from build123d import *

# Parameters (mm, degrees)
SKETCH1_W           = 220
SKETCH1_H           = 220
BOSS_EXTRUDE1_DEPTH = 70
SKETCH2_R           = 82.5
CUT_EXTRUDE1_DEPTH  = 171.587221092
M30_TAPPED_HOLE1_D  = 26.5
SKETCH7_R           = 22.5
CUT_EXTRUDE3_DEPTH  = 5
FILLET1_R           = 30
CHAMFER1_SIZE       = 3
SKETCH8_W           = 16
SKETCH8_H           = 87
CUT_EXTRUDE4_DEPTH  = 171.587221092


with BuildPart() as part:
    # Sketch1 → Boss-Extrude1 (new body)
    with BuildSketch(Plane.XY):
        Rectangle(SKETCH1_W, SKETCH1_H)
    extrude(amount=BOSS_EXTRUDE1_DEPTH)

    # Sketch2 → Cut-Extrude1 (cut, through all)
    with BuildSketch(Plane.XY.offset(70)):
        Circle(SKETCH2_R)
    extrude(amount=-CUT_EXTRUDE1_DEPTH, mode=Mode.SUBTRACT)

    # M30 Tapped Hole1 (through all)
    with Locations(Plane(origin=(110, 0, 0), x_dir=(0, 0, -1), z_dir=(1, 0, 0))):
        with Locations((-35, 0)):
            Hole(M30_TAPPED_HOLE1_D / 2)

    # Sketch7 → Cut-Extrude3 (cut)
    with BuildSketch(Plane.ZY.offset(110)):
        with Locations((35, 0)):
            Circle(SKETCH7_R)
    cut_extrude3 = extrude(amount=-CUT_EXTRUDE3_DEPTH, mode=Mode.SUBTRACT)

    # Mirror1: Cut-Extrude3 across plane
    add(cut_extrude3.mirror(Plane(origin=(0, 0, 0), x_dir=(0, 0, 1), z_dir=(1, 0, 0))), mode=Mode.SUBTRACT)

    # Fillet1
    fillet1_edges = [part.edges().sort_by_distance(p)[0] for p in [
        (-110, 110, 35),
        (110, 110, 35),
        (110, -110, 35),
        (-110, -110, 35),
    ]]
    fillet(fillet1_edges, radius=FILLET1_R)

    # Chamfer1
    chamfer1_edges = [part.edges().sort_by_distance(p)[0] for p in [
        (-82.5, 0, 0),
        (-82.5, 0, 70),
        (0, 110, 0),
        (0, 110, 70),
        (-110, 0, 0),
        (110, 0, 0),
        (0, -110, 0),
        (-101.213203436, 101.213203436, 0),
        (-101.213203436, -101.213203436, 0),
        (101.213203436, -101.213203436, 0),
        (101.213203436, 101.213203436, 0),
        (110, 0, 70),
        (-110, 0, 70),
        (0, -110, 70),
        (-101.213203436, 101.213203436, 70),
        (-101.213203436, -101.213203436, 70),
        (101.213203436, -101.213203436, 70),
        (101.213203436, 101.213203436, 70),
    ]]
    chamfer(chamfer1_edges, length=CHAMFER1_SIZE)

    # Sketch8 → Cut-Extrude4 (cut, through all)
    with BuildSketch(Plane(origin=(0, 0, 0), x_dir=(-1, 0, 0), z_dir=(0, 0, -1))):
        with Locations((0, -43.5)):
            Rectangle(SKETCH8_W, SKETCH8_H)
    extrude(amount=-CUT_EXTRUDE4_DEPTH, mode=Mode.SUBTRACT)


solid = part.part
Part model, mm, in its own coordinate system. A direction names the side the tool comes from. Give positions to 0.01 mm unless a question says otherwise; leave off trailing zeros. Order: outer loops, then holes, each group sorted by start corner. A loop starts at its lowest first (then second) coordinate and runs counter-clockwise, first axis right, second up. Notation, with made-up numbers: (33.5, 88) -> (70.5, 88) arc R14 ccw to (70.5, 109) -> close; hole circle Ø2 at (30, 52.25). An arc over 180 degrees is marked (long way). Use one line per item in the form item = value.
(1) Saw through at A-A (z = 35). Write the cut outline in (x, y).
Solution:
outline = (-110, -80) arc R30 ccw to (-80, -110) -> (80, -110) arc R30 ccw to (110, -80) -> (110, -22.5) -> (105, -22.5) -> (105, -13.25) -> (81.43, -13.25) arc R82.5 cw to (8, -82.11) -> (8, -87) -> (-8, -87) -> (-8, -82.11) arc R82.5 cw to (-81.43, -13.25) -> (-105, -13.25) -> (-105, -22.5) -> (-110, -22.5) -> close; (-110, 22.5) -> (-105, 22.5) -> (-105, 13.25) -> (-81.43, 13.25) arc R82.5 cw to (81.43, 13.25) -> (105, 13.25) -> (105, 22.5) -> (110, 22.5) -> (110, 80) arc R30 ccw to (80, 110) -> (-80, 110) arc R30 ccw to (-110, 80) -> close
(2) Saw through at B-B (x = 0). Write the cut outline in (y, z).
Solution:
outline = (-110, 3) -> (-107, 0) -> (-87, 0) -> (-87, 70) -> (-107, 70) -> (-110, 67) -> close; (82.5, 3) -> (85.5, 0) -> (107, 0) -> (110, 3) -> (110, 67) -> (107, 70) -> (85.5, 70) -> (82.5, 67) -> close
(3) Drill centre lines: line 1 (Z direction, x = 97, y = 0); line 2 (Y direction, x = 2, z = 46); line 3 (X direction, y = 73.5, z = 54.5). Where is each one in solid material? Low to high. Write a range as from..to.
Solution:
line_1 = 0..21.75, 48.25..70
line_2 = -110..-87, 82.48..110
line_3 = -110..-37.47, 37.47..110
(4) Tool access for faces 5 (the face through (-8, -85, 35)), 6 (the face through (100.979, -101.445, 35.448)): list every direction of +Z, -Z, +X, -X, +Y, -Y with a clear straight run to the whole face (end or side of a thin tool).
Solution:
face_5 = +Z, -Z
face_6 = +Z, -Z, +X, -Y
(5) Pull direction X, two halves, no side cores. Call faces 1 (the face through (-99.012, -99.435, 69.812)), 2 (the face through (100.979, 101.445, 35.448)), 3 (the face through (3.525, 82.57, 2.854)), 4 (the face through (8, -85, 35)): +X half, -X half, draft (parallel to the pull), parting line (faces both ways), or undercut.
Solution:
face_1 = -X half
face_2 = +X half
face_3 = undercut
face_4 = undercut
(6) Saw through at D-D (y = 9.5). Count the separate pieces of the cut face and the enclosed holes in it, then the cut area to 3 significant figures.
Solution:
separate_pieces = 4
enclosed_holes = 0
area = 2,630 mm²
(7) Flat gauge pins, fed straight in: P1, Ø1.5, axis at y = -84.5, z = 47.5, coming from the +X side; P2, Ø22.5, axis at y = 3, z = 36, coming from the +X side; P3, Ø5.5, axis at y = -85.5, z = 32.5, coming from the -X side. Where does each tip first touch, or does it go through?
Solution:
P1 = 109.76
P2 = 105
P3 = -109.87
(8) Saw through at C-C (z = 6). Write the cut outline in (x, y), then the cut area to 3 significant figures.
Solution:
outline = (-110, -80) arc R30 ccw to (-80, -110) -> (80, -110) arc R30 ccw to (110, -80) -> (110, 80) arc R30 ccw to (80, 110) -> (-80, 110) arc R30 ccw to (-110, 80) -> close; hole (-8, -87) -> (8, -87) -> (8, -82.11) arc R82.5 ccw (long way) to (-8, -82.11) -> close
area = 26,200 mm²
